```python
from build123d import *

# Parameters (mm, degrees)
BOSS_EXTRUDE1_DEPTH = 502
SKETCH2_R           = 5.5
CUT_EXTRUDE1_DEPTH  = 3
LPATTERN1_COUNT     = 2
LPATTERN1_PITCH     = 344


with BuildPart() as part:
    # Sketch1 → Boss-Extrude1 (new body)
    with BuildSketch(Plane.XY):
        with BuildLine():
            Line((0, 0), (30, 0))
            Line((30, 0), (30, 1))
            ThreePointArc((30, 1), (29.414213562, 2.414213562), (28, 3))
            Line((28, 3), (5, 3))
            ThreePointArc((5, 3), (3.585786438, 3.585786438), (3, 5))
            Line((3, 5), (3, 28))
            ThreePointArc((3, 28), (2.414213562, 29.414213562), (1, 30))
            Line((1, 30), (0, 30))
            Line((0, 30), (0, 0))
        make_face()
    extrude(amount=BOSS_EXTRUDE1_DEPTH)

    # Sketch2 → Cut-Extrude1 (cut)
    with BuildSketch(Plane.XZ):
        with Locations(Location((18.5, 482, 0), (0, 0, 270))):
            Circle(SKETCH2_R)
    cut_extrude1 = extrude(amount=-CUT_EXTRUDE1_DEPTH, mode=Mode.SUBTRACT)

    # LPattern1: Cut-Extrude1 ×2
    with Locations(*[(0, 0, -i * LPATTERN1_PITCH) for i in range(1, LPATTERN1_COUNT)]):
        add(cut_extrude1, mode=Mode.SUBTRACT)


solid = part.part
```
Source: CAD feature listing. Evaluate the final solid. Frame: model axes, mm. A direction names the side the tool comes from. Round coordinates to 2 decimals unless told otherwise and drop trailing zeros. Loops run counter-clockwise (first coordinate to the right, second up) from the corner with the lowest first, then second, coordinate; pieces in that order, holes last. Notation, with made-up numbers: M -21.75,47 L 0.25,47 A26 cw 0.25,76 Z; hole C 46,15 d4. An arc over 180 degrees is marked long. Use a Markdown table: item, result. Add a question column.
1. Cut plane D-D, the plane y = 21.75. Output: boundary loops of the cut face in (x, z), and give its area (3 significant figures).
2. Cut plane A-A, the plane x = 18.5. Output: boundary loops of the cut face in (y, z).
3. Pull-direction query (Z, two-part tool) for faces 3 (the cylindrical face through (15.2, 1.5, 142.4)), 4 (the flat face through (0, 15, 247)), 5 (the flat face through (2.7, 9.5, 502)); classes: +Z half, -Z half, draft (parallel to the pull), parting line (faces both ways), or undercut.
4. Ray query, line 1 along X through (y, z) = (0.75, 138); line 2 along Y through (x, z) = (24.25, 177.5); line 3 along X through (y, z) = (2, 482). Return the intervals inside material, ascending. Write a range as [from, to].
5. Cut plane C-C, the plane z = 482. Output: boundary loops of the cut face in (x, y).
6. Contact query for flat-ended pins moving along their axis: pin 1 (2 mm diameter, centred on y = 9.5, z = 133.5, fed in from +X); pin 2 (1 mm diameter, centred on x = 12.5, z = 119.5, fed in from +Y). Output: stop coordinate, or through.
7. Set-up query: faces 1 (the flat face through (15, 0, 247)), 2 (the flat face through (17, 3, 247)). Return all of +Z, -Z, +X, -X, +Y, -Y with unobstructed straight access to the full face (end or side cutting, diameter ignored); none if empty.
8. Cut plane B-B, the plane z = 194.5. Output: boundary loops of the cut face in (x, y).
Solution:
| question | item | result |
|---|---|---|
| 1 | outline | M 0,0 L 3,0 L 3,502 L 0,502 Z |
| 1 | area | 1,510 mm2 |
| 2 | outline | M 0,0 L 3,0 L 3,132.5 L 0,132.5 Z; M 0,143.5 L 3,143.5 L 3,476.5 L 0,476.5 Z; M 0,487.5 L 3,487.5 L 3,502 L 0,502 Z |
| 3 | face 3 | undercut |
| 3 | face 4 | draft |
| 3 | face 5 | +Z half |
| 4 | line 1 | x = [0, 13], [24, 30] |
| 4 | line 2 | y = [0, 3] |
| 4 | line 3 | x = [0, 13], [24, 29.73] |
| 5 | outline | M 0,0 L 13,0 L 13,3 L 5,3 A2 cw 3,5 L 3,28 A2 ccw 1,30 L 0,30 Z; M 24,0 L 30,0 L 30,1 A2 ccw 28,3 L 24,3 Z |
| 6 | pin 1 | stops at x = 3 |
| 6 | pin 2 | stops at y = 3 |
| 7 | face 1 | +Z, -Z, +X, -X, -Y |
| 7 | face 2 | +Z, -Z, +X, +Y |
| 8 | outline | M 0,0 L 30,0 L 30,1 A2 ccw 28,3 L 5,3 A2 cw 3,5 L 3,28 A2 ccw 1,30 L 0,30 Z |
